Job drawing, mm, ordinate dimensions from the low corner. One solid piece. Give positions to 0.01 mm unless a question says otherwise; leave off trailing zeros. Order: outer loops, then holes, each group sorted by start corner. A loop starts at its lowest first (then second) coordinate and runs counter-clockwise, first axis right, second up. Notation, with made-up numbers: (-21, 15.25) - (-12, 15.25) arc R29 cw to (-12, 47.25) - close; hole circle Ø10 at (51, -25). An arc over 180 degrees is marked (long way). Use one line per item in the form item = value. Start each with the question number.
1. Pull direction X, two halves, no side cores. Call the marked faces 1, 2 and 3: +X half, -X half, draft (parallel to the pull), parting line (faces both ways), or undercut.
2. Band-saw the part on A-A, the plane z = 30. List the corners of the cut face in (x, y), plus the area to 3 significant figures.
3. Band-saw the part on B-B, the plane z = 4.5. List the corners of the cut face in (x, y), plus the area to 3 significant figures.
4. Pin check, flat tip, straight feed: P1, Ø4, axis at x = 10, y = 12.5, coming from the -Z side. Stop position of the tip, or through.
5. Band-saw the part on C-C, the plane x = 2.5. List the corners of the cut face in (y, z).
6. Drill centre lines: line 1 (Y direction, x = 7.5, z = 32.25); line 2 (X direction, y = 13.03, z = 30.5); line 3 (Y direction, x = 5.5, z = 24.5). Where is each one in solid material? Low to high.
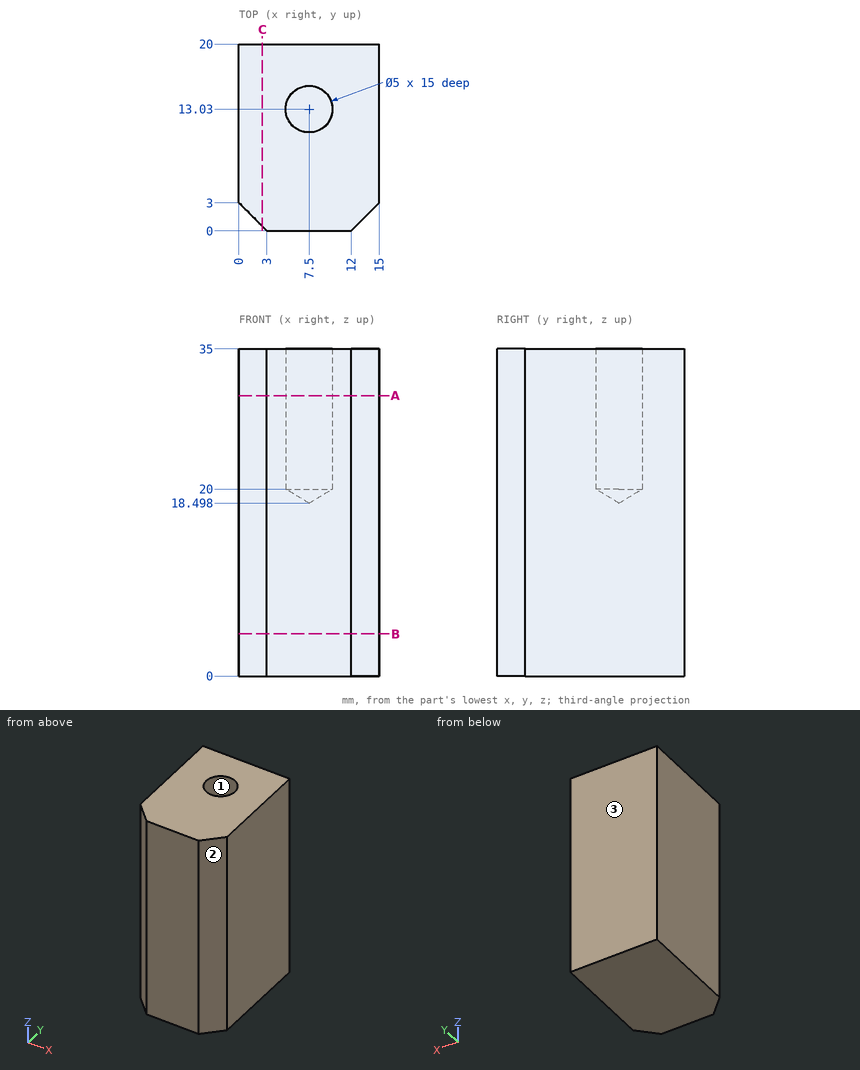
From the geometry:
q1.face_1 = undercut
q1.face_2 = +X half
q1.face_3 = draft
q2.outline = (0, 3) - (3, 0) - (12, 0) - (15, 3) - (15, 20) - (0, 20) - close; hole circle Ø5 at (7.5, 13.03)
q2.area = 271 mm²
q3.outline = (0, 3) - (3, 0) - (12, 0) - (15, 3) - (15, 20) - (0, 20) - close
q3.area = 291 mm²
q4.P1 = 0
q5.outline = (0.5, 0) - (20, 0) - (20, 35) - (0.5, 35) - close
q6.line_1 = 0 to 10.53, 15.53 to 20
q6.line_2 = 0 to 5, 10 to 15
q6.line_3 = 0 to 11.53, 14.53 to 20
